```python
from build123d import *

# Parameters (mm, degrees)
SKETCH_2_R               = 6.25
CUT_EXTRUDE_1_DEPTH      = 137.304805491
PATTERN_CIRCULAR_1_COUNT = 6
CHAMFER_1_SIZE           = 1


with BuildPart() as part:
    # 草图1 → 旋转1 (revolve)
    with BuildSketch(Plane.XY, mode=Mode.PRIVATE) as revolve_1_sk:
        Polygon((0, 0), (0, 95), (13, 95), (13, 45), (23, 45), (23, 30), (13, 30), (13, 0), align=None)
    revolve(revolve_1_sk.sketch.rotate(Axis((0, 0, 0), (1, 0, 0)), 90), axis=Axis((0, 0, 0), (1, 0, 0)))

    # 草图2 → 切除-拉伸1 (cut, through all)
    with BuildSketch(Plane.ZY):
        with Locations((0, 80)):
            Circle(SKETCH_2_R)
    cut_extrude_1 = extrude(amount=-CUT_EXTRUDE_1_DEPTH, mode=Mode.SUBTRACT)

    # 阵列(圆周)1: 切除-拉伸1 ×6 about axis
    pattern_circular_1_axis = Axis((0, 0, 0), (1, 0, 0))
    for i in range(1, PATTERN_CIRCULAR_1_COUNT):
        add(cut_extrude_1.rotate(pattern_circular_1_axis, i * 360 / PATTERN_CIRCULAR_1_COUNT), mode=Mode.SUBTRACT)

    # 倒角1
    chamfer_1_edges = [part.edges().sort_by_distance(p)[0] for p in [
        (23, 0, -30),
        (23, 0, -45),
        (13, 0, -95),
        (0, 0, -95),
    ]]
    chamfer(chamfer_1_edges, length=CHAMFER_1_SIZE)


solid = part.part
```
Check sheet for the modelled part. Datum: model origin and axes. Units: mm. A direction names the side the tool comes from. Round coordinates to 2 decimals unless told otherwise and drop trailing zeros. Loops run counter-clockwise (first coordinate to the right, second up) from the corner with the lowest first, then second, coordinate; pieces in that order, holes last. Notation, with made-up numbers: (85.5, -26) - (134.5, -26) arc R20 cw to (134.5, 2) - close; hole circle Ø7 at (-9.75, 39). An arc over 180 degrees is marked (long way). Write item = value, one per line. Start each with the question number.
Q1. Section check A-A (z = 0). Record the boundary of the cut face in (x, y), plus the area to 3 significant figures.
Q2. Section check D-D (y = -40). Count the separate pieces of the cut face and the enclosed holes in it, plus the area to 3 significant figures.
Q3. Section check C-C (x = 5.5). Record the boundary of the cut face in (y, z).
Q4. Depth check by flat-ended pin: P1, Ø11, axis at y = 40, z = 69.28, coming from the +X side; P2, Ø10, axis at x = 15.5, z = 5.5, coming from the +Y side; P3, Ø1, axis at y = 12.5, z = 36, coming from the -X side; P4, Ø12, axis at x = 8.5, y = 24.5, coming from the +Z side. Enter the tip coordinate at first touch or a pass-through.
Q5. Access from +Z, -Z, +X, -X, +Y, -Y to the whole of each face (thin tool, end or side, straight path). Record for faces 1 (the face through (6.409, 35.776, -64.676)), 2 (the face through (13, 0, 0)).
Q6. Thickness scan on L1, parallel to Y at x = 1, z = 70.5; L2, parallel to X at y = 81.5, z = -26; L3, parallel to Z at x = 2.75, y = 1.5. Record the ranges inside material, lowest first.
Q7. Section check B-B (y = 0). Record the boundary of the cut face in (x, z).
Q8. Release check for a two-part mould opening along Y. For faces 3 (the face through (6.41, 35.78, 73.89)), 4 (the face through (6.58, 92.74, -20.59)), 5 (the face through (0, -1, 1)), 6 (the face through (6.4, 86.2, -0.8)) record: pulls with the +Y half, pulls with the -Y half, needs draft (parallel to the pull), parting line crosses it, or undercut.
Derived:
q1.outline = (0, -94) - (1, -95) - (12, -95) - (13, -94) - (13, -86.25) - (0, -86.25) - close; (0, -73.75) - (13, -73.75) - (13, -45) - (22, -45) - (23, -44) - (23, -31) - (22, -30) - (13, -30) - (13, 30) - (22, 30) - (23, 31) - (23, 44) - (22, 45) - (13, 45) - (13, 73.75) - (0, 73.75) - close; (0, 86.25) - (13, 86.25) - (13, 94) - (12, 95) - (1, 95) - (0, 94) - close
q1.area = 2,440 mm^2
q2.separate_pieces = 3
q2.enclosed_holes = 0
q2.area = 2,320 mm^2
q3.outline = circle Ø190 at (0, 0); hole circle Ø12.5 at (-80, 0); hole circle Ø12.5 at (-40, -69.28); hole circle Ø12.5 at (-40, 69.28); hole circle Ø12.5 at (40, -69.28); hole circle Ø12.5 at (40, 69.28); hole circle Ø12.5 at (80, 0)
q4.P1 = through
q4.P2 = 94.98
q4.P3 = 0
q4.P4 = 93.18
q5.face_1 = +X, -X
q5.face_2 = +X
q6.L1 = -63.68 to -46.13, -33.87 to 33.87, 46.13 to 63.68
q6.L2 = 0 to 13
q6.L3 = -94.99 to 94.99
q7.outline = (0, -94) - (1, -95) - (12, -95) - (13, -94) - (13, -45) - (22, -45) - (23, -44) - (23, -31) - (22, -30) - (13, -30) - (13, 30) - (22, 30) - (23, 31) - (23, 44) - (22, 45) - (13, 45) - (13, 94) - (12, 95) - (1, 95) - (0, 94) - close
q8.face_3 = undercut
q8.face_4 = parting line crosses it
q8.face_5 = needs draft
q8.face_6 = undercut
